Can you work these out from the model? Positions are in its coordinate system, mm. Face numbers are marked on the shaded views. A direction names the side the tool comes from. Round coordinates to 2 decimals unless told otherwise and drop trailing zeros. Order: outer loops, then holes, each group sorted by start corner. A loop starts at its lowest first (then second) coordinate and runs counter-clockwise, first axis right, second up. Notation, with made-up numbers: (34.5, -18) -> (74.5, -18) arc R21 ccw to (74.5, -10) -> close; hole circle Ø3 at (78, 40). An arc over 180 degrees is marked (long way). One line per item, written item: value.
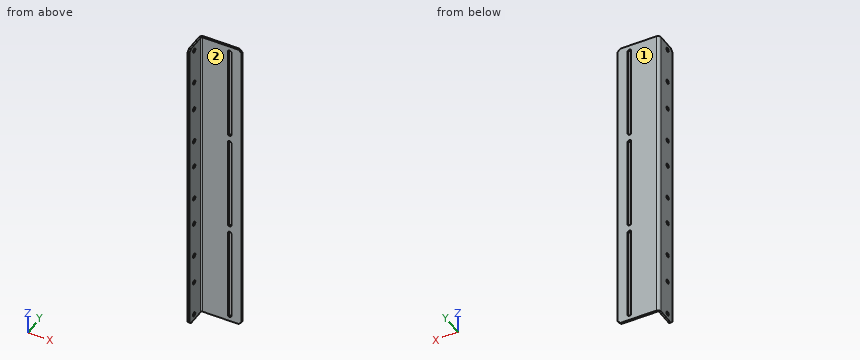
```python
from build123d import *

# Parameters (mm, degrees)
EXTRUDE_1_DEPTH     = 515
SKETCH_3_R          = 3.5
CUT_EXTRUDE_1_DEPTH = 515
CHAMFER_1_SIZE      = 5
CUT_EXTRUDE_2_DEPTH = 515


with BuildPart() as part:
    # 草图1 → 凸台-拉伸1 (new body)
    with BuildSketch(Plane.XY):
        with BuildLine():
            Line((0, 0), (-65, 0))
            ThreePointArc((-65, 0), (-68.535533906, -1.464466094), (-70, -5))
            Line((-70, -5), (-70, -40))
            Line((-70, -40), (-67, -40))
            Line((-67, -40), (-67, -5))
            ThreePointArc((-67, -5), (-66.414213562, -3.585786438), (-65, -3))
            Line((-65, -3), (0, -3))
            Line((0, -3), (0, 0))
        make_face()
    extrude(amount=EXTRUDE_1_DEPTH)

    # 草图3 → 切除-拉伸1 (cut)
    with BuildSketch(Plane.ZY.offset(70)):
        with Locations((10, -25)):
            Circle(SKETCH_3_R)
        with Locations((70, -25)):
            Circle(SKETCH_3_R)
        with Locations((287.5, -25)):
            Circle(SKETCH_3_R)
        with Locations((180, -25)):
            Circle(SKETCH_3_R)
        with Locations((120, -25)):
            Circle(SKETCH_3_R)
        with Locations((227.5, -25)):
            Circle(SKETCH_3_R)
        with Locations(Location((445, -25, 0), (0, 0, 180))):
            Circle(SKETCH_3_R)
        with Locations(Location((505, -25, 0), (0, 0, 180))):
            Circle(SKETCH_3_R)
        with Locations(Location((395, -25, 0), (0, 0, 180))):
            Circle(SKETCH_3_R)
        with Locations(Location((335, -25, 0), (0, 0, 180))):
            Circle(SKETCH_3_R)
    extrude(amount=-CUT_EXTRUDE_1_DEPTH, mode=Mode.SUBTRACT)

    # 倒角1
    chamfer_1_edges = [part.edges().sort_by_distance(p)[0] for p in [
        (-68.5, -40, 0),
        (0, -1.5, 515),
        (-68.5, -40, 515),
        (0, -1.5, 0),
    ]]
    chamfer(chamfer_1_edges, length=CHAMFER_1_SIZE)

    # 草图4 → 切除-拉伸2 (cut)
    with BuildSketch(Plane(origin=(0, 0, 0), x_dir=(1, 0, 0), z_dir=(0, 1, 0))):
        with BuildLine():
            Line((-17, -10.5), (-17, -164.5))
            ThreePointArc((-17, -164.5), (-20, -167.5), (-23, -164.5))
            Line((-23, -164.5), (-23, -10.5))
            ThreePointArc((-23, -10.5), (-20, -7.5), (-17, -10.5))
        make_face()
        with BuildLine():
            Line((-17, -180.5), (-17, -334.5))
            ThreePointArc((-17, -334.5), (-20, -337.5), (-23, -334.5))
            Line((-23, -334.5), (-23, -180.5))
            ThreePointArc((-23, -180.5), (-20, -177.5), (-17, -180.5))
        make_face()
        with BuildLine():
            Line((-17, -504.5), (-17, -350.5))
            ThreePointArc((-17, -350.5), (-20, -347.5), (-23, -350.5))
            Line((-23, -350.5), (-23, -504.5))
            ThreePointArc((-23, -504.5), (-20, -507.5), (-17, -504.5))
        make_face()
    extrude(amount=-CUT_EXTRUDE_2_DEPTH, mode=Mode.SUBTRACT)


solid = part.part
```
Q1. On a 3-axis mill with a long thin cutter (end or side, diameter ignored), from which of +Z, -Z, +X, -X, +Y, -Y can I reach the whole of each face in a straight line? I mean the marked faces 1 and 2. Say none if no direction works.
Answers below:
face 1: +Z, -Z, +X, -X, +Y
face 2: +Z, -Z, +X, -Y
Q2. Please list where these lines run through material, in increasing order: line 1 along Y through (x, z) = (-28.5, 456); line 2 along X through (y, z) = (-10, 199); line 3 along Y through (x, z) = (-69.15, 287.5).
Answers below:
line 1: -3 to 0
line 2: -70 to -67
line 3: -40 to -28.5, -21.5 to -2.21
Q3. I want a section at A-A on z = 468.5. List the corners of the cut face in (x, y) for me.
Answers below:
outline: (-70, -40) -> (-67, -40) -> (-67, -5) arc R2 cw to (-65, -3) -> (-23, -3) -> (-23, 0) -> (-65, 0) arc R5 ccw to (-70, -5) -> close; (-17, -3) -> (0, -3) -> (0, 0) -> (-17, 0) -> close
Q4. I want a section at C-C on y = -10.5. List the corners of the cut face in (x, z) for me.
Answers below:
outline: (-70, 0) -> (-67, 0) -> (-67, 515) -> (-70, 515) -> close
Q5. Will these pins go through, and if not, where does the flat tip stop? pin 1 Ø5.5 at (y, z) = (-25, 445) entering from +X; pin 2 Ø8 at (y, z) = (-25, 227.5) entering from +X; pin 3 Ø3.5 at (y, z) = (-1, 269) entering from -X; pin 4 Ø3 at (x, z) = (-40.5, 339) entering from -Y.
Answers below:
pin 1: through
pin 2: x = -67
pin 3: x = -69.47
pin 4: y = -3
Q6. I want a section at B-B on x = -11.5. List the corners of the cut face in (y, z) for me, plus the area to 4 significant figures.
Answers below:
outline: (-3, 0) -> (0, 0) -> (0, 515) -> (-3, 515) -> close
area: 1,545 mm^2
